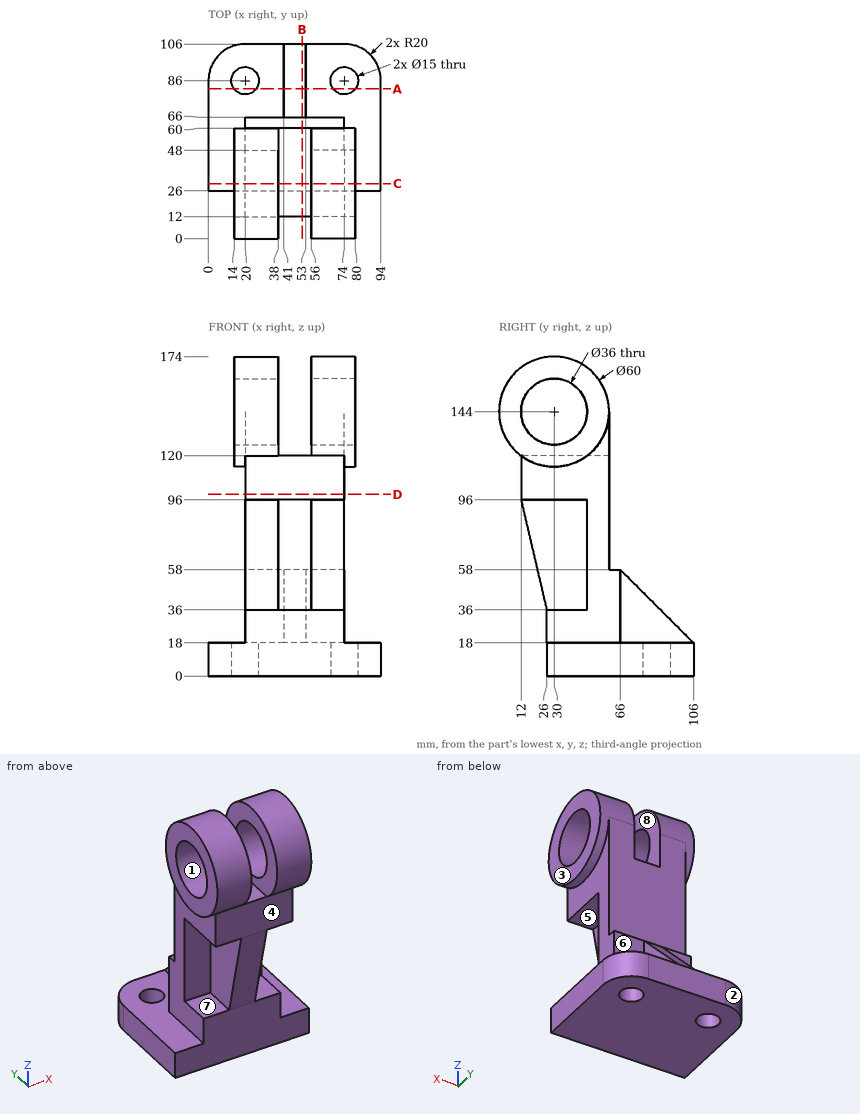
Check sheet for the drawn part. Datum: minimum x, y, z corner. Units: mm. A direction names the side the tool comes from. Give positions to 0.01 mm unless a question says otherwise; leave off trailing zeros. Loops run counter-clockwise (first coordinate to the right, second up) from the corner with the lowest first, then second, coordinate; pieces in that order, holes last. Notation, with made-up numbers: M 52.25,64.25 L 94.25,64.25 A22 ccw 94.25,75.25 Z; hole C -38,-35 d8. An arc over 180 degrees is marked long. Answer as CSV lines item,"result".
Item 1: Sectioned sample at A-A, the plane y = 81.5. Enter the section's corners in (x, z).
Reply:
outline,"M 0,0 L 14,0 L 14,18 L 0,18 Z; M 26,0 L 68,0 L 68,18 L 53,18 L 53,42.5 L 41,42.5 L 41,18 L 26,18 Z; M 80,0 L 94,0 L 94,18 L 80,18 Z"
Item 2: Sectioned sample at D-D, the plane z = 99. Enter the section's corners in (x, y), then the cut area to 3 significant figures.
Reply:
outline,"M 20,12 L 74,12 L 74,60 L 20,60 Z"
area,"2,590 mm^2"
Item 3: Scan lines: L1, parallel to Z at x = 31, y = 30; L2, parallel to Y at x = 33, z = 144; L3, parallel to Z at x = 74.5, y = 34.5. Record each from-to range of solid material in increasing order.
Reply:
L1,"0 to 36, 96 to 126, 162 to 174"
L2,"0 to 12, 48 to 60"
L3,"0 to 18, 114.34 to 126.57, 161.43 to 173.66"
Item 4: Set-up check for the marked faces 4, 5, 6, 7 and 8: record each of +Z, -Z, +X, -X, +Y, -Y from which the full face is reachable in a straight line by a thin tool's end or side.
Reply:
face 4,"-Z, +X, -X, -Y"
face 5,"+X, -Y"
face 6,"+Z, +X, +Y"
face 7,"-X, -Y"
face 8,"+Z, +Y, -Y"
Item 5: Sectioned sample at C-C, the plane y = 30. State how many separate pieces and enclosed holes the cut face has, then the cut area to 3 significant figures.
Reply:
separate pieces,"3"
enclosed holes,"0"
area,"5,980 mm^2"
Item 6: Draft check along Y on the marked faces 1, 2 and 3. Enter one of: pulls with the +Y half, pulls with the -Y half, needs draft (parallel to the pull), parting line crosses it, or undercut.
Reply:
face 1,"undercut"
face 2,"pulls with the +Y half"
face 3,"needs draft"
Item 7: Depth check by flat-ended pin: pin 1 Ø12 at (y, z) = (37.5, 58) entering from +X; pin 2 Ø12 at (x, z) = (58.5, 113) entering from -Y; pin 3 Ø23 at (x, z) = (26, 32) entering from +Y. Enter the tip coordinate at first touch or a pass-through.
Reply:
pin 1,"x = 56"
pin 2,"y = 12"
pin 3,"y = 66"
Item 8: Sectioned sample at B-B, the plane x = 51. Enter the section's corners in (y, z).
Reply:
outline,"M 12,96 L 26,36 L 26,0 L 106,0 L 106,18 L 66,58 L 60,58 L 60,120 L 12,120 Z"
